Here's the drawing with two shaded views (mm, measured from the low corner). I have some questions. Give positions to 0.01 mm unless a question says otherwise; leave off trailing zeros. Write each loop counter-clockwise with the first axis right and the second up, starting at its lowest first coordinate (ties: lowest second). Pieces come first, ordered by that corner, then holes.
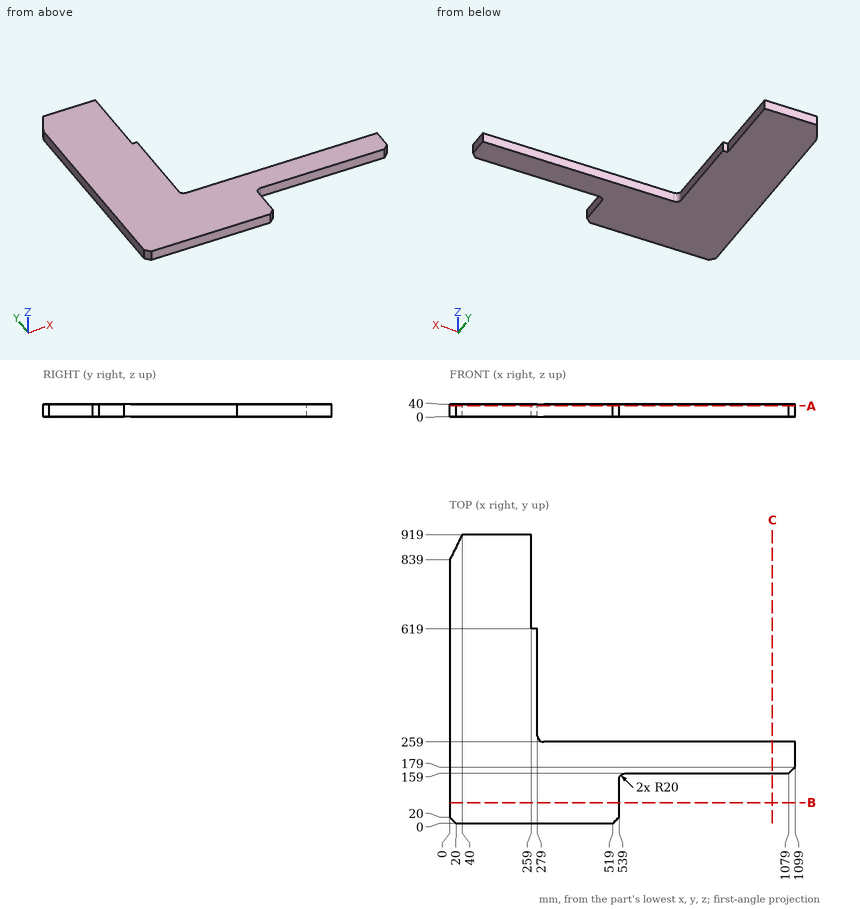
1) Please list where these lines run through material, in increasing order: L1, parallel to X at y = 93.5, z = 4; L2, parallel to X at y = 348, z = 15; L3, parallel to Y at x = 707, z = 15.
Values follow:
L1: x = 0 to 539
L2: x = 0 to 279
L3: y = 159 to 259
2) Suppose I cut it at C-C on x = 1027. Write out the boundary of the cut face in (y, z), plus the area to 3 significant figures.
Values follow:
outline: (159, 0) - (259, 0) - (259, 40) - (159, 40) - close
area: 4,000 mm2
3) For pin 1 Ø3 at (y, z) = (802.5, 13.5) entering from +X; pin 2 Ø3 at (x, z) = (980.5, 5.5) entering from -Y; pin 3 Ø3 at (x, y) = (503, 170) entering from -Z; pin 4 Ø6 at (x, z) = (266, 14) entering from +Y, each with a flat end and sliding along its axis, tell me the tip position at first contact or that it passes through.
Values follow:
pin 1: stops at x = 259
pin 2: stops at y = 159
pin 3: stops at z = 0
pin 4: stops at y = 619
4) Suppose I cut it at B-B on y = 66. Write out the boundary of the cut face in (x, z).
Values follow:
outline: (0, 0) - (539, 0) - (539, 40) - (0, 40) - close
5) Suppose I cut it at A-A on z = 34. Write out the boundary of the cut face in (x, y).
Values follow:
outline: (0, 20) - (20, 0) - (519, 0) - (539, 20) - (539, 139) arc R20 cw to (559, 159) - (1079, 159) - (1099, 179) - (1099, 259) - (299, 259) arc R20 cw to (279, 279) - (279, 619) - (259, 619) - (259, 919) - (40, 919) - (0, 839) - close
